Job drawing, mm, ordinate dimensions from the low corner. One solid piece. Give positions to 0.01 mm unless a question says otherwise; leave off trailing zeros. Write each loop counter-clockwise with the first axis right and the second up, starting at its lowest first coordinate (ties: lowest second). Pieces come first, ordered by that corner, then holes. Notation, with made-up numbers: (-21, 26.25) - (35, 26.25) arc R22 ccw to (35, 48.25) - close; hole circle Ø9 at (-4.5, -28). An arc over 180 degrees is marked (long way). Put each result on its own line as item: value. Start each with the question number.
1. Cut at B-B on y = 11. List the corners of the cut face in (x, z), and give its area (3 significant figures).
2. Cut at D-D on x = 14.5. List the corners of the cut face in (y, z).
3. Cut at A-A on z = 12.5. List the corners of the cut face in (x, y), and give its area (4 significant figures).
4. Cut at C-C on x = 87.5. List the corners of the cut face in (y, z), and give its area (3 significant figures).
5. Wall check: line 1 (X direction, y = 20, z = 12.5); line 2 (Z direction, x = 12.5, y = 15.5); line 3 (X direction, y = 28.5, z = 10.25). Give the ranges that are in metal, low to high.
6. Drop flat-ended pins along their axis: pin 1 (8 mm diameter, centred on x = 62.5, z = 12.5, fed in from -Y); pin 2 (4 mm diameter, centred on x = 37.5, z = 12.5, fed in from -Y). Give the stop position or say it passes through.
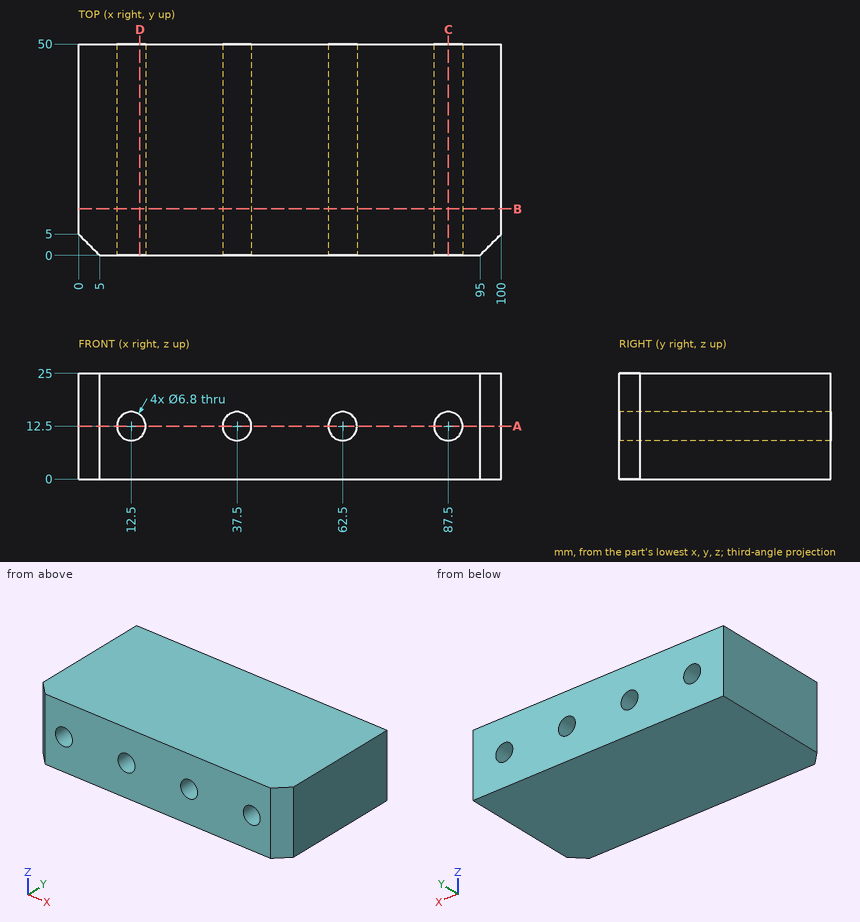
Report:
1. outline: (0, 0) - (100, 0) - (100, 25) - (0, 25) - close; hole circle Ø6.8 at (12.5, 12.5); hole circle Ø6.8 at (37.5, 12.5); hole circle Ø6.8 at (62.5, 12.5); hole circle Ø6.8 at (87.5, 12.5)
1. area: 2,350 mm²
2. outline: (0, 0) - (50, 0) - (50, 9.75) - (0, 9.75) - close; (0, 15.25) - (50, 15.25) - (50, 25) - (0, 25) - close
3. outline: (0, 5) - (5, 0) - (9.1, 0) - (9.1, 50) - (0, 50) - close; (15.9, 0) - (34.1, 0) - (34.1, 50) - (15.9, 50) - close; (40.9, 0) - (59.1, 0) - (59.1, 50) - (40.9, 50) - close; (65.9, 0) - (84.1, 0) - (84.1, 50) - (65.9, 50) - close; (90.9, 0) - (95, 0) - (100, 5) - (100, 50) - (90.9, 50) - close
3. area: 3,615 mm²
4. outline: (0, 0) - (50, 0) - (50, 9.1) - (0, 9.1) - close; (0, 15.9) - (50, 15.9) - (50, 25) - (0, 25) - close
4. area: 910 mm²
5. line 1: x = 0 to 9.1, 15.9 to 34.1, 40.9 to 59.1, 65.9 to 84.1, 90.9 to 100
5. line 2: z = 0 to 9.1, 15.9 to 25
5. line 3: x = 0 to 9.95, 15.05 to 34.95, 40.05 to 59.95, 65.05 to 84.95, 90.05 to 100
6. pin 1: stops at y = 0
6. pin 2: passes through
